Geometry: see drawing. Coordinates: mm, zero at the bounding-box minimum. A direction names the side the tool comes from. Coordinates: 2 decimals unless noted, no trailing zeros. Write each loop counter-clockwise with the first axis right and the second up, starting at its lowest first coordinate (ties: lowest second). Pieces come first, ordered by that corner, then holes. Notation, with made-up numbers: (29.25, 80.5) - (37.25, 80.5) arc R22 cw to (37.25, 112.5) - close; hole circle Ø8 at (79.25, 28). An arc over 180 degrees is marked (long way). One line per question, with ' | ' between items. Start each with the question number.
Q1. Cut plane D-D, the plane z = 3.75. Return loops of the section in (x, y).
Q2. Draft query along Y for the marked faces 1, 2 and 3. Return one class per face: +Y half, -Y half, draft (parallel to the pull), parting line (faces both ways), or undercut.
Q3. Cut plane C-C, the plane x = 22. Return loops of the section in (y, z), plus the area to 3 significant figures.
Q4. Contact query for flat-ended pins moving along their axis: P1, Ø8, axis at x = 15.5, y = 37.5, coming from the -Z side; P2, Ø2.5, axis at y = 36.5, z = 8.5, coming from the -X side; P3, Ø1.5, axis at y = 34, z = 7, coming from the +X side. Output: stop coordinate, or through.
Q5. Access query for the marked faces 4, 5, 6 and 7. Directions: +Z, -Z, +X, -X, +Y, -Y. A direction counts if a zero-diameter tool reaches every point of the face in a straight line with its end or side. Return the directions, or none.
Q6. Cut plane B-B, the plane x = 12. Return loops of the section in (y, z), plus the area to 3 significant figures.
Q7. Line query: line 1 (X direction, y = 36.5, z = 9); line 2 (Y direction, x = 8, z = 11.25); line 3 (Y direction, x = 28.5, z = 6.5). Output: solid intervals per line, ascending.
Q8. Cut plane A-A, the plane z = 8.25. Return loops of the section in (x, y).
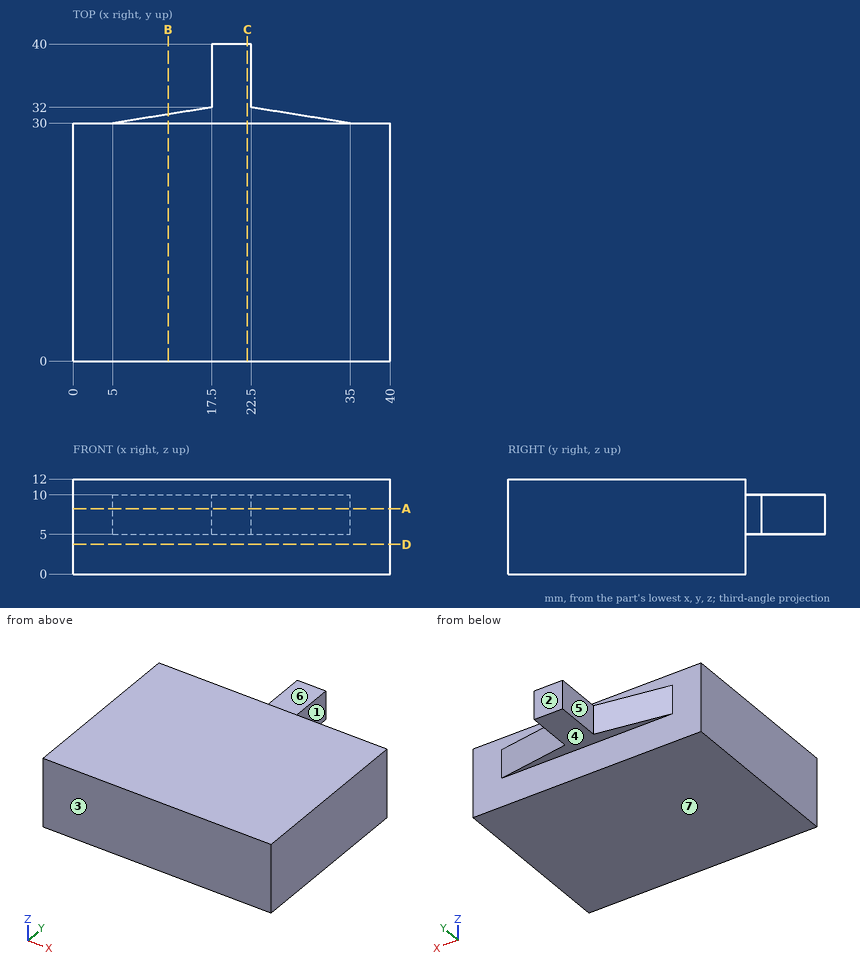
Reply:
1) outline: (0, 0) - (40, 0) - (40, 30) - (0, 30) - close
2) face 1: draft | face 2: +Y half | face 3: -Y half
3) outline: (0, 0) - (30, 0) - (30, 5) - (40, 5) - (40, 10) - (30, 10) - (30, 12) - (0, 12) - close | area: 410 mm^2
4) P1: stops at z = 5 | P2: stops at x = 17.5 | P3: stops at x = 22.5
5) face 4: -Z, +X, -X, +Y | face 5: +Z, -Z, -X, +Y | face 6: +Z, +X, -X, +Y | face 7: -Z, +X, -X, +Y, -Y
6) outline: (0, 0) - (30, 0) - (30, 5) - (31.12, 5) - (31.12, 10) - (30, 10) - (30, 12) - (0, 12) - close | area: 366 mm^2
7) line 1: x = 17.5 to 22.5 | line 2: y = 0 to 30 | line 3: y = 0 to 31.04
8) outline: (0, 0) - (40, 0) - (40, 30) - (35, 30) - (22.5, 32) - (22.5, 40) - (17.5, 40) - (17.5, 32) - (5, 30) - (0, 30) - close
